Geometry: final body of the model. Coordinates: model frame, mm. A direction names the side the tool comes from. Give positions to 0.01 mm unless a question says otherwise; leave off trailing zeros. Write each loop counter-clockwise with the first axis right and the second up, starting at its lowest first coordinate (ties: lowest second). Pieces come first, ordered by that corner, then holes. Notation, with made-up numbers: (-6.5, 19.25) -> (15.5, 19.25) arc R18 cw to (15.5, 29.25) -> close; hole circle Ø5 at (-20.5, 84.5). An arc over 180 degrees is marked (long way). Answer as a JSON object with one key per item and string values.
from build123d import *

# Parameters (mm, degrees)
EXTRUDE_1_DEPTH         = 50
SKETCH_3_R              = 23.75
CUT_EXTRUDE_1_DEPTH     = 116.956888541
HOLE_WIZARD_11_0_11_1_D = 11
HOLE_WIZARD_8_5_8_5_1_D = 8.5
CHAMFER_1_SIZE          = 3
FILLET_1_R              = 4
FILLET_2_R              = 12


with BuildPart() as part:
    # 草图1 → 凸台-拉伸1 (new, symmetric)
    with BuildSketch(Plane(origin=(0, 0, 0), x_dir=(0, 0, -1), z_dir=(1, 0, 0))):
        Polygon((-61, 85), (-61, 50.5), (-8, 50.5), (-8, -50.5), (-61, -50.5), (-61, -85), (-53, -85), (-53, -58.5), (0, -58.5), (0, 58.5), (-53, 58.5), (-53, 85), align=None)
    extrude(amount=EXTRUDE_1_DEPTH, both=True)

    # 草图3 → 切除-拉伸1 (cut, through all)
    with BuildSketch(Plane(origin=(0, 0, 0), x_dir=(-1, 0, 0), z_dir=(0, 0, -1))):
        with Locations(Location((0, 0, 0), (0, 0, 90))):
            Circle(SKETCH_3_R)
    extrude(amount=-CUT_EXTRUDE_1_DEPTH, mode=Mode.SUBTRACT)

    # Ø11.0 (11) 直径孔1 (through all)
    with Locations(Plane(origin=(0, 0, 0), x_dir=(-1, 0, 0), z_dir=(0, 0, -1))):
        with Locations((0, 0), (35, -35), (-35, 35), (-35, -35), (35, 35)):
            Hole(HOLE_WIZARD_11_0_11_1_D / 2)

    # Ø8.5 (8.5) 直径孔1 (through all)
    with Locations(Plane(origin=(0, 0, 53), x_dir=(-1, 0, 0), z_dir=(0, 0, -1))):
        with Locations((-35, -73), (0, -73), (35, -73), (35, 73), (0, 73), (-35, 73)):
            Hole(HOLE_WIZARD_8_5_8_5_1_D / 2)

    # 倒角1
    chamfer_1_edges = [part.edges().sort_by_distance(p)[0] for p in [
        (-50, -85, 57),
        (-50, 85, 57),
        (50, -85, 57),
        (50, 85, 57),
    ]]
    chamfer(chamfer_1_edges, length=CHAMFER_1_SIZE)

    # 圆角1
    fillet_1_edges = [part.edges().sort_by_distance(p)[0] for p in [
        (0, 58.5, 53),
        (0, -58.5, 53),
        (0, -50.5, 8),
        (0, 50.5, 8),
    ]]
    fillet(fillet_1_edges, radius=FILLET_1_R)

    # 圆角2
    fillet_2_edges = [part.edges().sort_by_distance(p)[0] for p in [
        (0, 58.5, 0),
        (0, -58.5, 0),
        (0, -50.5, 61),
        (0, 50.5, 61),
    ]]
    fillet(fillet_2_edges, radius=FILLET_2_R)


solid = part.part
Q1. Cut plane C-C (x = -22). Return the cut outline in (y, z), and give its area (3 significant figures).
Values:
{"outline": "(-85, 53) -> (-62.5, 53) arc R4 cw to (-58.5, 49) -> (-58.5, 12) arc R12 ccw to (-46.5, 0) -> (-8.95, 0) -> (-8.95, 8) -> (-46.5, 8) arc R4 cw to (-50.5, 12) -> (-50.5, 49) arc R12 ccw to (-62.5, 61) -> (-85, 61) -> close; (8.95, 0) -> (46.5, 0) arc R12 ccw to (58.5, 12) -> (58.5, 49) arc R4 cw to (62.5, 53) -> (85, 53) -> (85, 61) -> (62.5, 61) arc R12 ccw to (50.5, 49) -> (50.5, 12) arc R4 cw to (46.5, 8) -> (8.95, 8) -> close", "area": "1,950 mm²"}
Q2. Set-up query: faces 4 (the flat face through (1, -79, 53)), 5 (the cylindrical face through (-0.7, 59.703, 51.859)), 6 (the flat face through (1, -50.5, 30)). Return all of +Z, -Z, +X, -X, +Y, -Y with unobstructed straight access to the full face (end or side cutting, diameter ignored); none if empty.
Values:
{"face 4": "-Z, +X, -X, -Y", "face 5": "-Z, +X, -X, +Y", "face 6": "+Z, +X, -X"}
Q3. First-contact query: P1, Ø11, axis at x = -7, y = -69, coming from the -Z side; P2, Ø11, axis at x = 12, z = 22, coming from the -Y side; P3, Ø5, axis at x = 4, z = 50, coming from the -Y side. Flat tips, straight axial feed; report the tip coordinate or a pass-through.
Values:
{"P1": "z = 53", "P2": "y = -58.5", "P3": "y = -60.56"}
Q4. Material intervals for L1, parallel to Y at x = -35, z = 1; L2, parallel to Y at x = 18.5, z = 30.5; L3, parallel to Y at x = -35, z = 3.5, sorted ascending. Write a range as from..to.
Values:
{"L1": "-51.3..-40.5, -29.5..29.5, 40.5..51.3", "L2": "-58.5..-50.5, 50.5..58.5", "L3": "-54.97..-40.5, -29.5..29.5, 40.5..54.97"}
Q5. Mould query, pull axis X, two halves, no side actions, for faces 1 (the flat face through (1, 79, 53)), 2 (the flat face through (-50, 0, 6)), 3 (the cylindrical face through (31.63, 70.41, 57.06)). Classes: pulls with the +X half, pulls with the -X half, needs draft (parallel to the pull), parting line crosses it, or undercut.
Values:
{"face 1": "needs draft", "face 2": "pulls with the -X half", "face 3": "undercut"}
Q6. Cut plane B-B (y = 0). Return the cut outline in (x, z), and give its area (3 significant figures).
Values:
{"outline": "(-50, 0) -> (-23.75, 0) -> (-23.75, 8) -> (-50, 8) -> close; (23.75, 0) -> (50, 0) -> (50, 8) -> (23.75, 8) -> close", "area": "420 mm²"}
Q7. Cut plane A-A (z = 22.5). Return the cut outline in (x, y), and give its area (3 significant figures).
Values:
{"outline": "(-50, -58.5) -> (50, -58.5) -> (50, -50.5) -> (-50, -50.5) -> close; (-50, 50.5) -> (50, 50.5) -> (50, 58.5) -> (-50, 58.5) -> close", "area": "1,600 mm²"}
Q8. Cut plane D-D (y = -35). Return the cut outline in (x, z), and give its area (3 significant figures).
Values:
{"outline": "(-50, 0) -> (-40.5, 0) -> (-40.5, 8) -> (-50, 8) -> close; (-29.5, 0) -> (29.5, 0) -> (29.5, 8) -> (-29.5, 8) -> close; (40.5, 0) -> (50, 0) -> (50, 8) -> (40.5, 8) -> close", "area": "624 mm²"}
